Part print with two shaded views. Sizes in mm from the minimum x, y, z corner. A direction names the side the tool comes from. Round coordinates to 2 decimals unless told otherwise and drop trailing zeros. Write each loop counter-clockwise with the first axis right and the second up, starting at its lowest first coordinate (ties: lowest second). Pieces come first, ordered by that corner, then holes. Notation, with made-up numbers: M -38.5,68 L -26.5,68 A15 cw -26.5,82 Z; hole C -14.5,-24.5 d7. An arc over 180 degrees is marked long. One line per question, with ' | ' between items. Start each with the question number.
1) Tool access for the marked faces 1, 2, 3 and 4: list every direction of +Z, -Z, +X, -X, +Y, -Y with a clear straight run to the whole face (end or side of a thin tool).
2) Saw through at A-A (x = 4). List the corners of the cut face in (y, z), plus the area to 3 significant figures.
3) Mould opens along X. For the marked faces 5, 6, 7 and 8 say: pulls with the +X half, pulls with the -X half, needs draft (parallel to the pull), parting line crosses it, or undercut.
4) Saw through at B-B (y = 7.5). List the corners of the cut face in (x, z).
5) Drop flat-ended pins along their axis: pin 1 Ø1 at (y, z) = (12.5, 8) entering from -X; pin 2 Ø3 at (x, z) = (4, 16.8) entering from +Y; pin 3 Ø1.2 at (x, z) = (7.5, 15.5) entering from -Y; pin 4 Ø2.5 at (x, y) = (3, 2.5) entering from +Z. Give the stop position or say it passes through.
6) Saw through at D-D (x = 0.75). List the corners of the cut face in (y, z).
7) Wall check: probe 1 along Z at (x, y) = (4, 13.15); probe 2 along Z at (x, y) = (4, 10.3); probe 3 along Z at (x, y) = (5, 6.5). Give the ranges that are in metal, low to high. Write a range as [from, to].
8) Saw through at C-C (z = 16.8). List the corners of the cut face in (x, y).
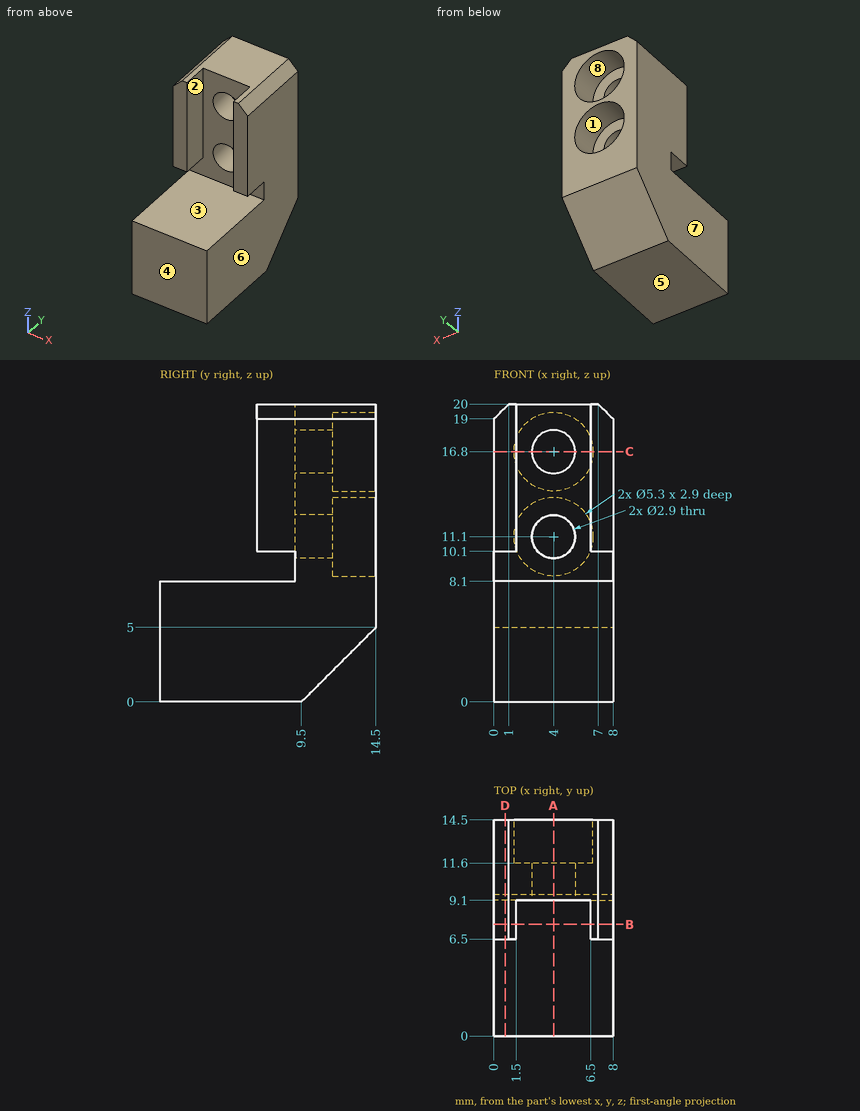
Answer key:
1) face 1: +Y | face 2: +Z, -Y | face 3: +X, -X, -Y | face 4: +Z, -Z, +X, -X, -Y
2) outline: M 0,0 L 9.5,0 L 14.5,5 L 14.5,8.45 L 11.6,8.45 L 11.6,9.65 L 9.1,9.65 L 9.1,8.1 L 0,8.1 Z; M 9.1,12.55 L 11.6,12.55 L 11.6,13.75 L 14.5,13.75 L 14.5,14.15 L 11.6,14.15 L 11.6,15.35 L 9.1,15.35 Z; M 9.1,18.25 L 11.6,18.25 L 11.6,19.45 L 14.5,19.45 L 14.5,20 L 9.1,20 Z | area: 124 mm2
3) face 5: needs draft | face 6: pulls with the +X half | face 7: pulls with the -X half | face 8: undercut
4) outline: M 0,0 L 8,0 L 8,8.1 L 0,8.1 Z; M 0,10.1 L 1.5,10.1 L 1.5,20 L 1,20 L 0,19 Z; M 6.5,10.1 L 8,10.1 L 8,19 L 7,20 L 6.5,20 Z
5) pin 1: stops at x = 0 | pin 2: stops at y = 11.6 | pin 3: stops at y = 6.5 | pin 4: stops at z = 8.1
6) outline: M 0,0 L 9.5,0 L 14.5,5 L 14.5,19.75 L 6.5,19.75 L 6.5,10.1 L 9.1,10.1 L 9.1,8.1 L 0,8.1 Z
7) probe 1: z = [3.65, 8.45], [13.75, 14.15], [19.45, 20] | probe 2: z = [0.8, 9.65], [12.55, 15.35], [18.25, 20] | probe 3: z = [0, 8.1]
8) outline: M 0,6.5 L 1.5,6.5 L 1.5,9.1 L 2.55,9.1 L 2.55,11.6 L 1.35,11.6 L 1.35,14.5 L 0,14.5 Z; M 5.45,9.1 L 6.5,9.1 L 6.5,6.5 L 8,6.5 L 8,14.5 L 6.65,14.5 L 6.65,11.6 L 5.45,11.6 Z
